from build123d import *

# Parameters (mm, degrees)
SKETCH1_R                                       = 25
BOSS_EXTRUDE1_DEPTH                             = 8
SKETCH2_R                                       = 17.5
CUT_EXTRUDE1_DEPTH                              = 5.5
SKETCH3_R                                       = 3
CUT_EXTRUDE2_DEPTH                              = 4
CSK_FOR_M3_FLAT_HEAD_MACHINE_SCREW1_D           = 3.4
CSK_FOR_M3_FLAT_HEAD_MACHINE_SCREW1_CSINK_D     = 6.3
CSK_FOR_M3_FLAT_HEAD_MACHINE_SCREW1_CSINK_ANGLE = 90


with BuildPart() as part:
    # Sketch1 → Boss-Extrude1 (new body)
    with BuildSketch(Plane(origin=(0, 0, 0), x_dir=(1, 0, 0), z_dir=(0, 1, 0))):
        with Locations(Location((0, 0, 0), (0, 0, 270))):
            Circle(SKETCH1_R)
    extrude(amount=BOSS_EXTRUDE1_DEPTH)

    # Sketch2 → Cut-Extrude1 (cut)
    with BuildSketch(Plane(origin=(0, 8, 0), x_dir=(1, 0, 0), z_dir=(0, 1, 0))):
        with Locations(Location((0, 0, 0), (0, 0, 270))):
            Circle(SKETCH2_R)
    extrude(amount=-CUT_EXTRUDE1_DEPTH, mode=Mode.SUBTRACT)

    # Sketch3 → Cut-Extrude2 (cut)
    with BuildSketch(Plane.XZ):
        with Locations(Location((0, -9, 0), (0, 0, 270))):
            Circle(SKETCH3_R)
        with Locations(Location((-6.363961031, -6.363961031, 0), (0, 0, 270))):
            Circle(SKETCH3_R)
        with Locations(Location((-9, 0, 0), (0, 0, 270))):
            Circle(SKETCH3_R)
        with Locations(Location((-6.363961031, 6.363961031, 0), (0, 0, 270))):
            Circle(SKETCH3_R)
        with Locations(Location((0, 9, 0), (0, 0, 270))):
            Circle(SKETCH3_R)
        with Locations(Location((6.363961031, 6.363961031, 0), (0, 0, 270))):
            Circle(SKETCH3_R)
        with Locations(Location((9, 0, 0), (0, 0, 270))):
            Circle(SKETCH3_R)
        with Locations(Location((6.363961031, -6.363961031, 0), (0, 0, 270))):
            Circle(SKETCH3_R)
    extrude(amount=-CUT_EXTRUDE2_DEPTH, mode=Mode.SUBTRACT)

    # CSK for M3 Flat Head Machine Screw1 (through all)
    with Locations(Plane(origin=(0, 0, 0), x_dir=(-1, 0, 0), z_dir=(0, -1, 0))):
        with Locations((20.5, 0), (0, 20.5), (-20.5, 0), (0, -20.5)):
            CounterSinkHole(CSK_FOR_M3_FLAT_HEAD_MACHINE_SCREW1_D / 2, CSK_FOR_M3_FLAT_HEAD_MACHINE_SCREW1_CSINK_D / 2, counter_sink_angle=CSK_FOR_M3_FLAT_HEAD_MACHINE_SCREW1_CSINK_ANGLE)


solid = part.part
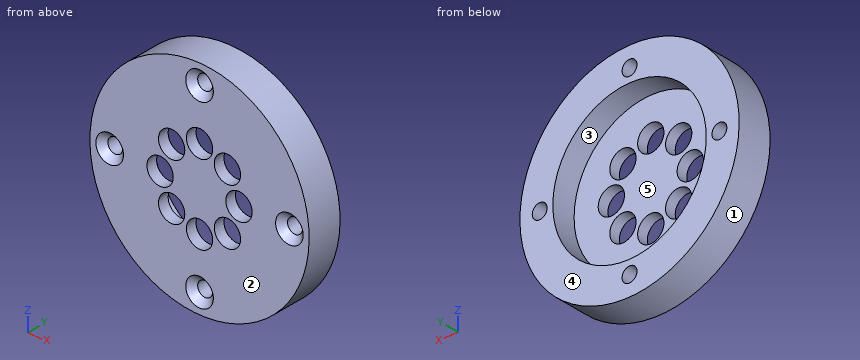
Model file for the job. Use its own axes, mm. Face numbers are marked on the shaded views. A direction names the side the tool comes from. Coordinates: 2 decimals unless noted, no trailing zeros. Write each loop counter-clockwise with the first axis right and the second up, starting at its lowest first coordinate (ties: lowest second). Pieces come first, ordered by that corner, then holes. Notation, with made-up numbers: (57, 8.5) -> (102, 8.5) arc R8 cw to (102, 17.5) -> close; hole circle Ø1 at (-9.5, 63). An arc over 180 degrees is marked (long way). One line per item, written item: value. Start each with the question number.
1) Slice it at B-B on y = 5.75. Write the cut outline in (x, z), then the cut area to 3 significant figures.
2) Slice it at D-D on z = -11. Write the cut outline in (x, y), then the cut area to 3 significant figures.
3) Which spindle directions (+Z, -Z, +X, -X, +Y, -Y) get a long thin tool onto all of the face, cutting with end or side? Do the marked faces 4 and 5. Say none if no direction does.
4) Pull direction Z, two halves, no side cores. Call the marked faces 1, 2 and 3: +Z half, -Z half, draft (parallel to the pull), parting line (faces both ways), or undercut.
5) Probe probe 1 along X at (y, z) = (1.25, -4.5); probe 2 along X at (y, z) = (0.75, 2); probe 3 along Z at (x, y) = (5, 2.25). List the from-to ranges inside material, lowest first.
6) Flat gauge pins, fed straight in: pin 1 Ø1 at (y, z) = (5.5, 11.5) entering from -X; pin 2 Ø3 at (x, y) = (18.5, 1) entering from +Z; pin 3 Ø8 at (x, z) = (-9, 0) entering from +Y. Where does each tip first touch, or does it go through?
7) Slice it at A-A on x = 0. Write the cut outline in (y, z), then the cut area to 3 significant figures.
8) Slice it at C-C on z = 8. Write the cut outline in (x, y), then the cut area to 3 significant figures.
Answers follow:
1. outline: circle Ø50 at (0, 0); hole circle Ø3.4 at (-20.5, 0); hole circle Ø35 at (0, 0); hole circle Ø3.4 at (0, -20.5); hole circle Ø3.4 at (0, 20.5); hole circle Ø3.4 at (20.5, 0)
1. area: 965 mm2
2. outline: (-22.45, 0) -> (-2.24, 0) -> (-2.24, 2.5) -> (-13.61, 2.5) -> (-13.61, 8) -> (-22.45, 8) -> close; (2.24, 0) -> (22.45, 0) -> (22.45, 8) -> (13.61, 8) -> (13.61, 2.5) -> (2.24, 2.5) -> close
2. area: 198 mm2
3. face 4: +Z, -Z, +X, -X, +Y
3. face 5: +Y
4. face 1: parting line
4. face 2: draft
4. face 3: undercut
5. probe 1: -24.59 to -8.71, -4.01 to 4.01, 8.71 to 24.59
5. probe 2: -24.92 to -21.83, -19.17 to -11.24, -6.76 to 6.76, 11.24 to 19.17, 21.83 to 24.92
5. probe 3: -24.49 to -9.04, -3.69 to 3.69, 9.04 to 24.49
6. pin 1: x = -22.45
6. pin 2: z = 18.33
6. pin 3: y = 2.5
7. outline: (0, -25) -> (8, -25) -> (8, -22.2) -> (1.45, -22.2) -> (0, -23.65) -> close; (0, -17.35) -> (1.45, -18.8) -> (8, -18.8) -> (8, -17.5) -> (2.5, -17.5) -> (2.5, -12) -> (0, -12) -> close; (0, -6) -> (2.5, -6) -> (2.5, 6) -> (0, 6) -> close; (0, 12) -> (2.5, 12) -> (2.5, 17.5) -> (8, 17.5) -> (8, 18.8) -> (1.45, 18.8) -> (0, 17.35) -> close; (0, 23.65) -> (1.45, 22.2) -> (8, 22.2) -> (8, 25) -> (0, 25) -> close
7. area: 119 mm2
8. outline: (-23.69, 0) -> (-8.88, 0) -> (-8.88, 2.5) -> (-15.56, 2.5) -> (-15.56, 8) -> (-23.69, 8) -> close; (-3.85, 0) -> (-2.83, 0) -> (-2.83, 2.5) -> (-3.85, 2.5) -> close; (2.83, 0) -> (3.85, 0) -> (3.85, 2.5) -> (2.83, 2.5) -> close; (8.88, 0) -> (23.69, 0) -> (23.69, 8) -> (15.56, 8) -> (15.56, 2.5) -> (8.88, 2.5) -> close
8. area: 168 mm2
